```python
from build123d import *

# Parameters (mm, degrees)
EXTRUDE_THIN1_DEPTH = 10


with BuildPart() as part:
    # Sketch2 → Extrude-Thin1 (new body)
    with BuildSketch(Plane.XY):
        with BuildLine():
            Line((-30.341760221, -69.425568872), (-30.341760221, -3.000568872))
            ThreePointArc((-30.341760221, -3.000568872), (-13.396760221, 13.944431128), (3.548239779, -3.000568872))
            Line((3.548239779, -3.000568872), (3.548239779, -69.425568872))
            ThreePointArc((3.548239779, -69.425568872), (-13.396760221, -86.370568872), (-30.341760221, -69.425568872))
        make_face()
        with BuildLine():
            Line((-28.341760221, -69.425568872), (-28.341760221, -3.000568872))
            ThreePointArc((-28.341760221, -3.000568872), (-13.396760221, 11.944431128), (1.548239779, -3.000568872))
            Line((1.548239779, -3.000568872), (1.548239779, -69.425568872))
            ThreePointArc((1.548239779, -69.425568872), (-13.396760221, -84.370568872), (-28.341760221, -69.425568872))
        make_face(mode=Mode.SUBTRACT)
    extrude(amount=EXTRUDE_THIN1_DEPTH)


solid = part.part
```
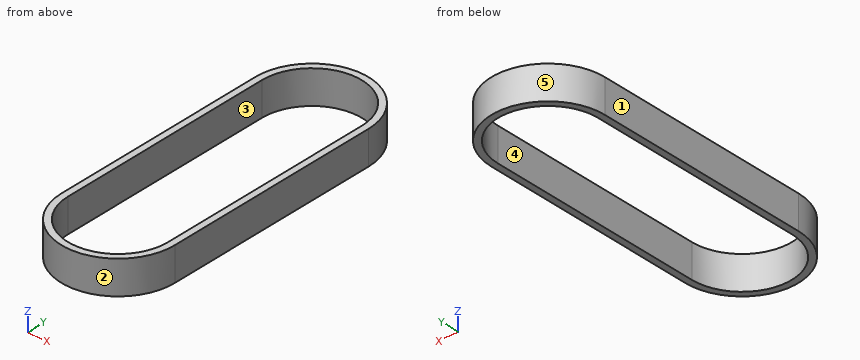
CAD build for the part. Positions are in the model's coordinates, mm. Face numbers are marked on the shaded views. A direction names the side the tool comes from. Give positions to 0.01 mm unless a question says otherwise; leave off trailing zeros. Order: outer loops, then holes, each group sorted by start corner. A loop starts at its lowest first (then second) coordinate and runs counter-clockwise, first axis right, second up. Notation, with made-up numbers: M -4.75,32 L 2.25,32 A24 cw 2.25,53 Z; hole C 76,20 d9. An arc over 180 degrees is marked long. Put each result on its own line as item: value. Start each with the question number.
(1) Saw through at B-B, the plane z = 6. Write the cut outline in (x, y) (3 decimals), then the cut area to 3 significant figures.
(2) Drill centre lines: line 1 along X through (y, z) = (-44.5, 7); line 2 along Y through (x, z) = (-21.5, 5.5); line 3 along Y through (x, z) = (-17.5, 1.25). Where is each one in solid material? Low to high.
(3) Saw through at A-A, the plane y = -50. Write the cut outline in (x, z), then the cut area to 3 significant figures.
(4) Mould opens along Y. For the marked faces 1, 2 and 3 say: +Y half, -Y half, draft (parallel to the pull), parting line (faces both ways), or undercut.
(5) Flat gauge pin, fed straight in: pin 1 Ø1 at (x, z) = (-24, 7.5) entering from -Y. Where does the tip first touch, or does it go through?
(6) Saw through at C-C, the plane x = -9.5. Write the cut outline in (y, z), then the cut area to 3 significant figures.
(7) Which spindle directions (+Z, -Z, +X, -X, +Y, -Y) get a long thin tool onto all of the face, cutting with end or side? Do the marked faces 4 and 5. Say none if no direction does.
Check result:
1. outline: M -30.342,-69.426 A16.945 ccw 3.548,-69.426 L 3.548,-3.001 A16.945 ccw -30.342,-3.001 Z; hole M -28.342,-69.426 A14.945 ccw 1.548,-69.426 L 1.548,-3.001 A14.945 ccw -28.342,-3.001 Z
1. area: 466 mm2
2. line 1: x = -30.34 to -28.34, 1.55 to 3.55
2. line 2: y = -84.31 to -81.98, 9.56 to 11.88
2. line 3: y = -85.87 to -83.8, 11.37 to 13.44
3. outline: M -30.34,0 L -28.34,0 L -28.34,10 L -30.34,10 Z; M 1.55,0 L 3.55,0 L 3.55,10 L 1.55,10 Z
3. area: 40.0 mm2
4. face 1: draft
4. face 2: -Y half
4. face 3: undercut
5. pin 1: stops at y = -83.03
6. outline: M -85.92,0 L -83.85,0 L -83.85,10 L -85.92,10 Z; M 11.43,0 L 13.49,0 L 13.49,10 L 11.43,10 Z
6. area: 41.3 mm2
7. face 4: +Z, -Z
7. face 5: +Z, -Z, +Y
